```python
from build123d import *

# Parameters (mm, degrees)
SKETCH_1_R             = 8
EXTRUDE_1_DEPTH        = 38.5
SKETCH_2_W             = 5
SKETCH_2_H             = 16
CUT_EXTRUDE_1_DEPTH    = 24
SKETCH_3_R             = 5.1
CUT_EXTRUDE_2_DEPTH    = 24
CUT_EXTRUDE_3_DEPTH    = 41.969500851
HOLE_WIZARD_M8_1_D     = 6.8
HOLE_WIZARD_M8_1_DEPTH = 12
HOLE_WIZARD_M8_1_TIP   = 2.042926105


with BuildPart() as part:
    # 草图1 → 凸台-拉伸1 (new body)
    with BuildSketch(Plane.XY):
        Circle(SKETCH_1_R)
    extrude(amount=EXTRUDE_1_DEPTH)

    # 草图2 → 切除-拉伸1 (cut)
    with BuildSketch(Plane.XY.offset(38.5)):
        with Locations((6, 0)):
            Rectangle(SKETCH_2_W, SKETCH_2_H)
        with Locations((-6, 0)):
            Rectangle(SKETCH_2_W, SKETCH_2_H)
    extrude(amount=-CUT_EXTRUDE_1_DEPTH, mode=Mode.SUBTRACT)

    # 草图3 → 切除-拉伸2 (cut)
    with BuildSketch(Plane(origin=(3.5, 0, 0), x_dir=(0, 0, -1), z_dir=(1, 0, 0))):
        with Locations(Location((-30, 0, 0), (0, 0, 90))):
            Circle(SKETCH_3_R)
    extrude(amount=-CUT_EXTRUDE_2_DEPTH, mode=Mode.SUBTRACT)

    # 草图4 → 切除-拉伸3 (cut, through all)
    with BuildSketch(Plane(origin=(3.5, 0, 0), x_dir=(0, 0, -1), z_dir=(1, 0, 0))):
        with BuildLine():
            Line((-30, 8.5), (-30, 11))
            Line((-30, 11), (-45, 11))
            Line((-45, 11), (-45, -11))
            Line((-45, -11), (-30, -11))
            Line((-30, -11), (-30, -8.5))
            ThreePointArc((-30, -8.5), (-38.5, 0), (-30, 8.5))
        make_face()
    extrude(amount=-CUT_EXTRUDE_3_DEPTH, mode=Mode.SUBTRACT)

    # M8 螺纹孔1
    with Locations(Plane(origin=(0, 0, 0), x_dir=(-1, 0, 0), z_dir=(0, 0, -1))):
        with Locations((0, 0)):
            Hole(HOLE_WIZARD_M8_1_D / 2, depth=HOLE_WIZARD_M8_1_DEPTH)
            with Locations((0, 0, -(HOLE_WIZARD_M8_1_DEPTH + HOLE_WIZARD_M8_1_TIP / 2))):  # 118° drill point
                Cone(0, HOLE_WIZARD_M8_1_D / 2, HOLE_WIZARD_M8_1_TIP, mode=Mode.SUBTRACT)


solid = part.part
```
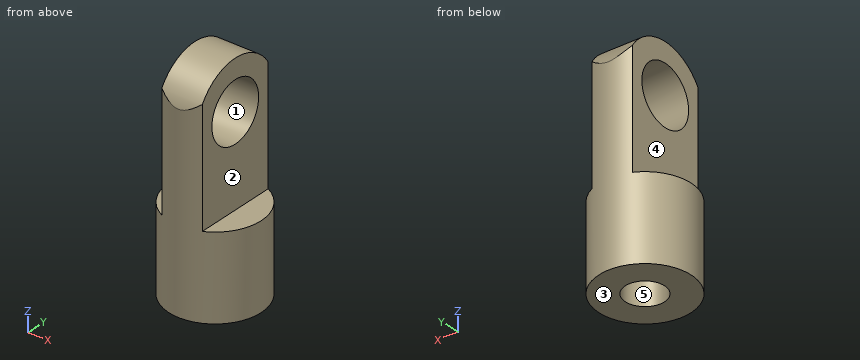
Geometry check sheet. Reference: the model listing, model coordinates, mm. Face numbers are marked on the shaded views. A direction names the side the tool comes from. Give positions to 0.01 mm unless a question says otherwise; leave off trailing zeros. Order: outer loops, then holes, each group sorted by start corner. A loop starts at its lowest first (then second) coordinate and runs counter-clockwise, first axis right, second up. Notation, with made-up numbers: (78.25, 57) - (108.25, 57) arc R18 cw to (108.25, 89) - close; hole circle Ø1 at (-19, -4). An arc over 180 degrees is marked (long way). Answer in a Markdown table with one row per item. Add a question column.
Q1. Cross-section at A-A, the plane z = 25.5. Enter the section's corners in (x, y).
Q2. Cross-section at B-B, the plane z = 7. Enter the section's corners in (x, y).
Q3. Cross-section at D-D, the plane z = 30. Enter the section's corners in (x, y).
Q4. Material ranges on probe 1 along X at (y, z) = (0.25, 5.5); probe 2 along X at (y, z) = (-1.5, 2.5), recorded low to high. Write a range as from..to.
Q5. Mould release check, pull along X, two halves, no side actions. Record for the marked faces 3, 4 and 5: pulls with the +X half, pulls with the -X half, needs draft (parallel to the pull), parting line crosses it, or undercut.
Q6. Tool access check on the marked faces 1 and 2. Record the directions out of +Z, -Z, +X, -X, +Y, -Y that give a thin tool (end or side, any length) a straight path to the whole face; none if there is none.
Q7. Gauge pin test, flat ends, axial feed: pin 1 (2 mm diameter, centred on x = -1, y = 2.5, fed in from -Z); pin 2 (4 mm diameter, centred on x = -5, z = 11, fed in from -Y); pin 3 (2 mm diameter, centred on x = -2.5, z = 29, fed in from +Y); pin 4 (7 mm diameter, centred on y = -1.5, z = 29, fed in from -X). Record the tip position at first contact, or that the pin passes through.
Q8. Cross-section at C-C, the plane y = 6. Enter the section's corners in (x, z).
Check values:
| question | item | result |
|---|---|---|
| 1 | outline | (-3.5, -7.19) arc R8 ccw to (3.5, -7.19) - (3.5, -2.4) - (-3.5, -2.4) - close; (-3.5, 2.4) - (3.5, 2.4) - (3.5, 7.19) arc R8 ccw to (-3.5, 7.19) - close |
| 2 | outline | circle Ø16 at (0, 0); hole circle Ø6.8 at (0, 0) |
| 3 | outline | (-3.5, -7.19) arc R8 ccw to (3.5, -7.19) - (3.5, -5.1) - (-3.5, -5.1) - close; (-3.5, 5.1) - (3.5, 5.1) - (3.5, 7.19) arc R8 ccw to (-3.5, 7.19) - close |
| 4 | probe 1 | x = -8..-3.39, 3.39..8 |
| 4 | probe 2 | x = -7.86..-3.05, 3.05..7.86 |
| 5 | face 3 | needs draft |
| 5 | face 4 | pulls with the -X half |
| 5 | face 5 | undercut |
| 6 | face 1 | +X, -X |
| 6 | face 2 | +Z, +X, +Y, -Y |
| 7 | pin 1 | stops at z = 0 |
| 7 | pin 2 | stops at y = -7.42 |
| 7 | pin 3 | stops at y = 7.86 |
| 7 | pin 4 | stops at x = -3.5 |
| 8 | outline | (-5.29, 0) - (5.29, 0) - (5.29, 14.5) - (3.5, 14.5) - (3.5, 36.02) - (-3.5, 36.02) - (-3.5, 14.5) - (-5.29, 14.5) - close |
